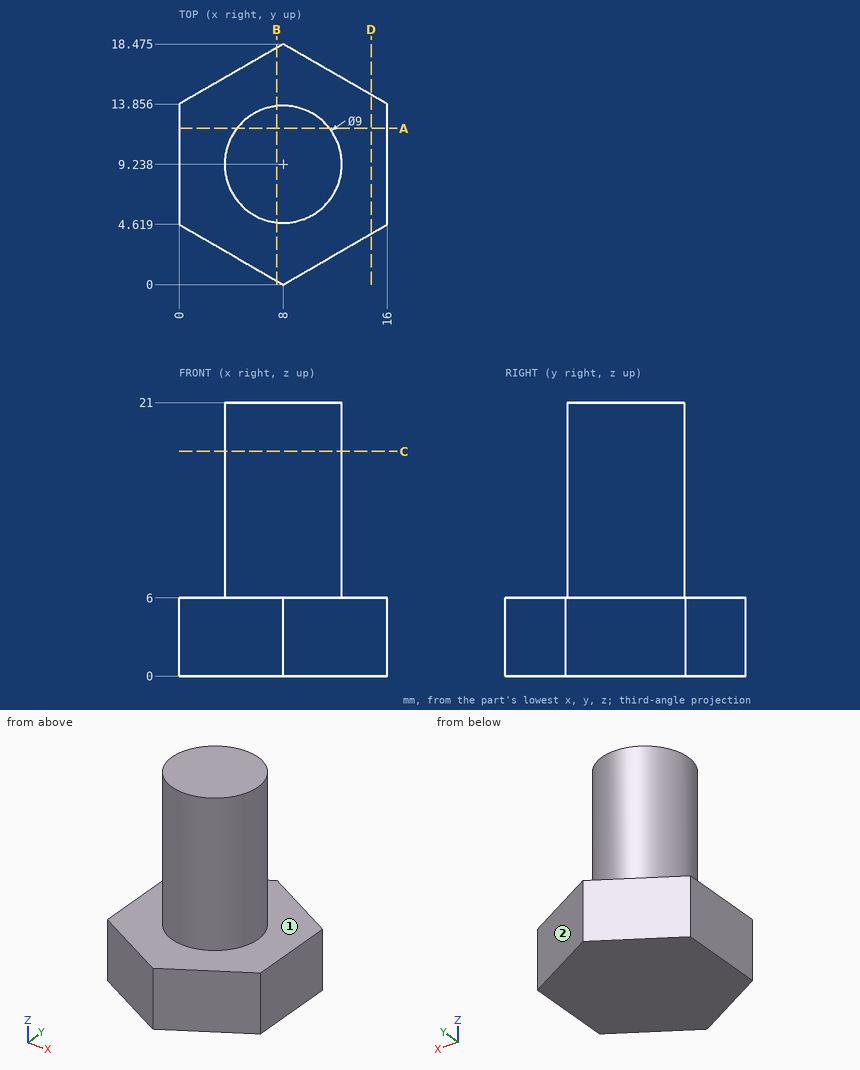
Input: dimensioned drawing with shaded views. Units: mm. Origin: part minimum x, y, z. A direction names the side the tool comes from. Round coordinates to 2 decimals unless told otherwise and drop trailing zeros. Order: outer loops, then holes, each group sorted by start corner. A loop starts at its lowest first (then second) coordinate and runs counter-clockwise, first axis right, second up. Notation, with made-up numbers: (4.25, -33) -> (29.25, -33) arc R26 cw to (29.25, 1) -> close; hole circle Ø2 at (11, 67). An arc over 180 degrees is marked (long way). One line per item, written item: value. Start each with the question number.
Q1. Pin query (flat end, axial travel): pin 1 (4 mm diameter, centred on x = 10.5, z = 13.5, fed in from +Y); pin 2 (1.5 mm diameter, centred on x = 8.5, y = 2.5, fed in from +Z); pin 3 (3 mm diameter, centred on x = 5, z = 6, fed in from +Y). Return the tip coordinate at first contact, or that it passes through.
Q2. Access query for the marked faces 1 and 2. Directions: +Z, -Z, +X, -X, +Y, -Y. A direction counts if a zero-diameter tool reaches every point of the face in a straight line with its end or side. Return the directions, or none.
Q3. Material intervals for probe 1 along Z at (x, y) = (3.25, 8.25); probe 2 along Y at (x, z) = (8, 11.25); probe 3 along X at (y, z) = (7.5, 13.25), sorted ascending.
Q4. Section query B-B (x = 7.5). Return the cut outline in (y, z) (1 decimal).
Q5. Section query D-D (x = 14.75). Return the cut outline in (y, z), plus the area to 3 significant figures.
Q6. Section query A-A (y = 12). Return the cut outline in (x, z).
Q7. Section query C-C (z = 17.25). Return the cut outline in (x, y).
Findings below:
1. pin 1: y = 13.71
1. pin 2: z = 6
1. pin 3: y = 17.61
2. face 1: +Z
2. face 2: +Z, -Z, +X, +Y
3. probe 1: 0 to 6
3. probe 2: 4.74 to 13.74
3. probe 3: 3.85 to 12.15
4. outline: (0.3, 0) -> (18.2, 0) -> (18.2, 6) -> (13.7, 6) -> (13.7, 21) -> (4.8, 21) -> (4.8, 6) -> (0.3, 6) -> close
5. outline: (3.9, 0) -> (14.58, 0) -> (14.58, 6) -> (3.9, 6) -> close
5. area: 64.1 mm²
6. outline: (0, 0) -> (16, 0) -> (16, 6) -> (11.55, 6) -> (11.55, 21) -> (4.45, 21) -> (4.45, 6) -> (0, 6) -> close
7. outline: circle Ø9 at (8, 9.24)
